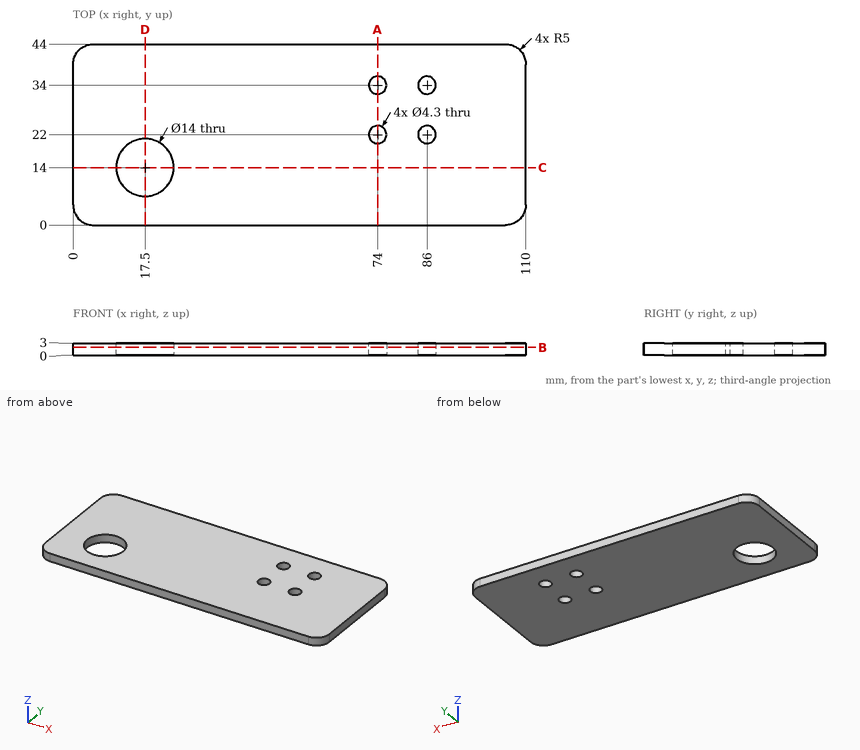
Geometry check sheet. Reference: drawing and pictorial views, mm from the part's lowest x, y, z. Round coordinates to 2 decimals unless told otherwise and drop trailing zeros. Order: outer loops, then holes, each group sorted by start corner. A loop starts at its lowest first (then second) coordinate and runs counter-clockwise, first axis right, second up.
Q1. Cross-section at C-C, the plane y = 14. Enter the section's corners in (x, z), plus the area to 3 significant figures.
Filled sheet:
outline: (0, 0) - (10.5, 0) - (10.5, 3) - (0, 3) - close; (24.5, 0) - (110, 0) - (110, 3) - (24.5, 3) - close
area: 288 mm2
Q2. Scan lines: L1, parallel to Y at x = 86, z = 2.1; L2, parallel to Y at x = 17.5, z = 0.9; L3, parallel to X at y = 17, z = 1.6. Record each from-to range of solid material in increasing order.
Filled sheet:
L1: y = 0 to 19.85, 24.15 to 31.85, 36.15 to 44
L2: y = 0 to 7, 21 to 44
L3: x = 0 to 11.18, 23.82 to 110
Q3. Cross-section at D-D, the plane x = 17.5. Enter the section's corners in (y, z), plus the area to 3 significant figures.
Filled sheet:
outline: (0, 0) - (7, 0) - (7, 3) - (0, 3) - close; (21, 0) - (44, 0) - (44, 3) - (21, 3) - close
area: 90.0 mm2
Q4. Cross-section at B-B, the plane z = 2. Enter the section's corners in (x, y).
Filled sheet:
outline: (0, 5) arc R5 ccw to (5, 0) - (105, 0) arc R5 ccw to (110, 5) - (110, 39) arc R5 ccw to (105, 44) - (5, 44) arc R5 ccw to (0, 39) - close; hole circle Ø14 at (17.5, 14); hole circle Ø4.3 at (74, 22); hole circle Ø4.3 at (74, 34); hole circle Ø4.3 at (86, 22); hole circle Ø4.3 at (86, 34)
Q5. Cross-section at A-A, the plane x = 74. Enter the section's corners in (y, z).
Filled sheet:
outline: (0, 0) - (19.85, 0) - (19.85, 3) - (0, 3) - close; (24.15, 0) - (31.85, 0) - (31.85, 3) - (24.15, 3) - close; (36.15, 0) - (44, 0) - (44, 3) - (36.15, 3) - close
